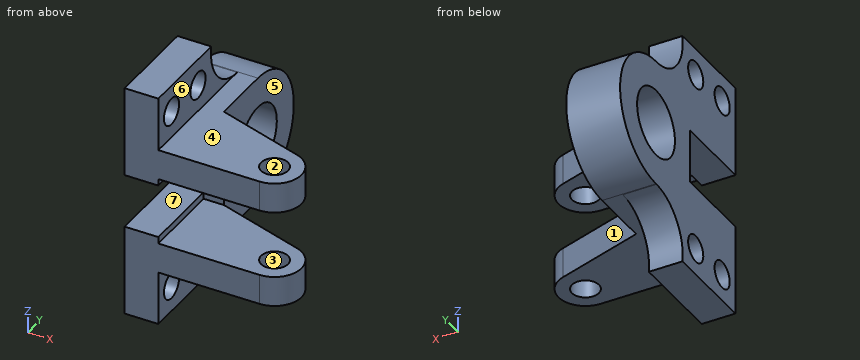
```python
from build123d import *

# Parameters (mm, degrees)
HUB_PROFILE_SKETCH_R    = 20
HUB_BOSS_DEPTH          = 16
ARM_PROFILE_SKETCH_R    = 8
ARM_BOSS_DEPTH          = 18
FLANGE_PROFILE_SKETCH_R = 8
FLANGE_BOSS_DEPTH       = 20
WEB_PROFILE_SKETCH_W    = 4
WEB_PROFILE_SKETCH_H    = 48
WEB_BOSS_DEPTH          = 20


with BuildPart() as part:
    # Hub Profile Sketch → Hub Boss (new, symmetric)
    with BuildSketch(Plane(origin=(0, 0, 0), x_dir=(0, 0, -1), z_dir=(1, 0, 0))):
        with BuildLine():
            Line((-38, 0), (-38, -36))
            Line((-38, -36), (38, -36))
            Line((38, -36), (38, 0))
            ThreePointArc((38, 0), (0, 38), (-38, 0))
        make_face()
        Circle(HUB_PROFILE_SKETCH_R, mode=Mode.SUBTRACT)
    extrude(amount=HUB_BOSS_DEPTH, both=True)

    # Arm Profile Sketch → Arm Boss (add)
    with BuildSketch(Plane.XY.offset(38)):
        with BuildLine():
            ThreePointArc((68.834711668, -52.747932498), (79.811911333, -70.446111196), (64, -84))
            Line((64, -84), (-16, -84))
            Line((-16, -84), (-16, -36))
            Line((-16, -36), (16, -36))
            Line((16, -36), (68.834711668, -52.747932498))
        make_face()
        with Locations((64, -68)):
            Circle(ARM_PROFILE_SKETCH_R, mode=Mode.SUBTRACT)
    arm_boss = extrude(amount=-ARM_BOSS_DEPTH)

    # Arm Mirror: Arm Boss across plane
    add(arm_boss.mirror(Plane.XY))

    # Flange Profile Sketch → Flange Boss (add)
    with BuildSketch(Plane.ZY.offset(16)):
        with BuildLine():
            ThreePointArc((70, -28), (47.777657825, -21.547691645), (38, -0.574800039))
            Line((38, -0.574800039), (38, -84))
            Line((38, -84), (70, -84))
            Line((70, -84), (70, -28))
        make_face()
        with Locations((54, -70)):
            Circle(FLANGE_PROFILE_SKETCH_R, mode=Mode.SUBTRACT)
        with Locations((54, -42)):
            Circle(FLANGE_PROFILE_SKETCH_R, mode=Mode.SUBTRACT)
    flange_boss = extrude(amount=-FLANGE_BOSS_DEPTH)

    # Flange Mirror: Flange Boss across plane
    add(flange_boss.mirror(Plane.XY))

    # Web Profile Sketch → Web Boss (add)
    with BuildSketch(Plane.ZY.offset(16)):
        with Locations((-18, -60)):
            Rectangle(WEB_PROFILE_SKETCH_W, WEB_PROFILE_SKETCH_H)
    web_boss = extrude(amount=-WEB_BOSS_DEPTH)

    # Web Mirror: Web Boss across plane
    add(web_boss.mirror(Plane.XY))


solid = part.part
```
Geometry check sheet. Reference: the model listing, model coordinates, mm. Face numbers are marked on the shaded views. A direction names the side the tool comes from. Coordinates: 2 decimals unless noted, no trailing zeros. Order: outer loops, then holes, each group sorted by start corner. A loop starts at its lowest first (then second) coordinate and runs counter-clockwise, first axis right, second up. Notation, with made-up numbers: (38, 2.25) - (68, 2.25) arc R13 cw to (68, 14.25) - close; hole circle Ø11 at (67.5, 1). An arc over 180 degrees is marked (long way). Use one line per item in the form item = value.
1. Scan lines: line 1 (Z direction, x = 37, y = -60.5); line 2 (X direction, y = -35, z = 27); line 3 (Y direction, x = -1, z = -54). Record each from-to range of solid material in increasing order.
Here are the results:
line_1 = -38 to -20, 20 to 38
line_2 = -16 to 16
line_3 = -84 to -78, -62 to -50, -34 to -25.59
2. Gauge pin test, flat ends, axial feed: pin 1 (4 mm diameter, centred on y = -32, z = 51.5, fed in from +X); pin 2 (14.5 mm diameter, centred on x = 29, y = -69, fed in from -Z); pin 3 (10 mm diameter, centred on x = 21.5, y = -59, fed in from +Z); pin 4 (21 mm diameter, centred on y = -70, z = 54, fed in from -X). Record the tip position at first contact, or that the pin passes through.
Here are the results:
pin_1 = 4
pin_2 = -38
pin_3 = 38
pin_4 = -16
3. Access from +Z, -Z, +X, -X, +Y, -Y to the whole of each face (thin tool, end or side, straight path). Record for the marked faces 5, 6 and 7.
Here are the results:
face_5 = +Z, -Z, +X, +Y
face_6 = +Z, +X, +Y, -Y
face_7 = +X, -X, -Y
4. Section check D-D (x = 8). Record the boundary of the cut face in (y, z).
Here are the results:
outline = (-84, -38) - (0, -38) arc R38 ccw to (0, 38) - (-84, 38) - (-84, 20) - (-36, 20) - (-36, -20) - (-84, -20) - close; hole circle Ø40 at (0, 0)
5. Section check A-A (x = 74). Record the boundary of the cut face in (y, z).
Here are the results:
outline = (-80.49, -38) - (-55.51, -38) - (-55.51, -20) - (-80.49, -20) - close; (-80.49, 20) - (-55.51, 20) - (-55.51, 38) - (-80.49, 38) - close
6. Section check C-C (z = 49). Record the boundary of the cut face in (x, y) (3 decimals), then the cut area to 3 significant figures.
Here are the results:
outline = (-16, -84) - (4, -84) - (4, -76.245) - (-16, -76.245) - close; (-16, -63.755) - (4, -63.755) - (4, -48.245) - (-16, -48.245) - close; (-16, -35.755) - (4, -35.755) - (4, -22.537) - (-16, -22.537) - close
area = 730 mm²
7. Draft check along Y on the marked faces 1, 2, 3 and 4. Enter one of: pulls with the +Y half, pulls with the -Y half, needs draft (parallel to the pull), parting line crosses it, or undercut.
Here are the results:
face_1 = pulls with the +Y half
face_2 = undercut
face_3 = undercut
face_4 = needs draft
8. Section check B-B (y = -68). State how many separate pieces and enclosed holes the cut face has, then the cut area to 3 significant figures.
Here are the results:
separate_pieces = 6
enclosed_holes = 0
area = 3,700 mm²
